Source: three-view drawing plus pictorial views. Frame: mm from the lowest corner of the part. A direction names the side the tool comes from. Give positions to 0.01 mm unless a question says otherwise; leave off trailing zeros. Write each loop counter-clockwise with the first axis right and the second up, starting at its lowest first coordinate (ties: lowest second). Pieces come first, ordered by that corner, then holes.
Q1. Pin query (flat end, axial travel): pin 1 (1.5 mm diameter, centred on x = 1.5, z = 3.5, fed in from -Y); pin 2 (5 mm diameter, centred on x = 2.5, y = 1, fed in from -Z); pin 3 (0.5 mm diameter, centred on y = 4.5, z = 7, fed in from -X). Return the tip coordinate at first contact, or that it passes through.
Q2. Line query: L1, parallel to X at y = 5.5, z = 7.25; L2, parallel to Y at x = 1, z = 1.5; L3, parallel to Y at x = 6, z = 2.5. Output: solid intervals per line, ascending.
Q3. Cut plane D-D on x = 7.5. Return the cut outline in (y, z), plus the area to 3 significant figures.
Q4. Cut plane B-B on y = 5. Return the cut outline in (x, z).
Q5. Cut plane A-A on z = 5. Return the cut outline in (x, y).
Q6. Reachability of the marked faces 1 and 2 from +Z, -Z, +X, -X, +Y, -Y: full face, straight path, thin tool, end or side. Return the list, or none.
Q7. Draft query along Y for the marked faces 3, 4 and 5. Return one class per face: pulls with the +Y half, pulls with the -Y half, needs draft (parallel to the pull), parting line crosses it, or undercut.
Q8. Cut plane C-C on x = 2.75. Return the cut outline in (y, z).
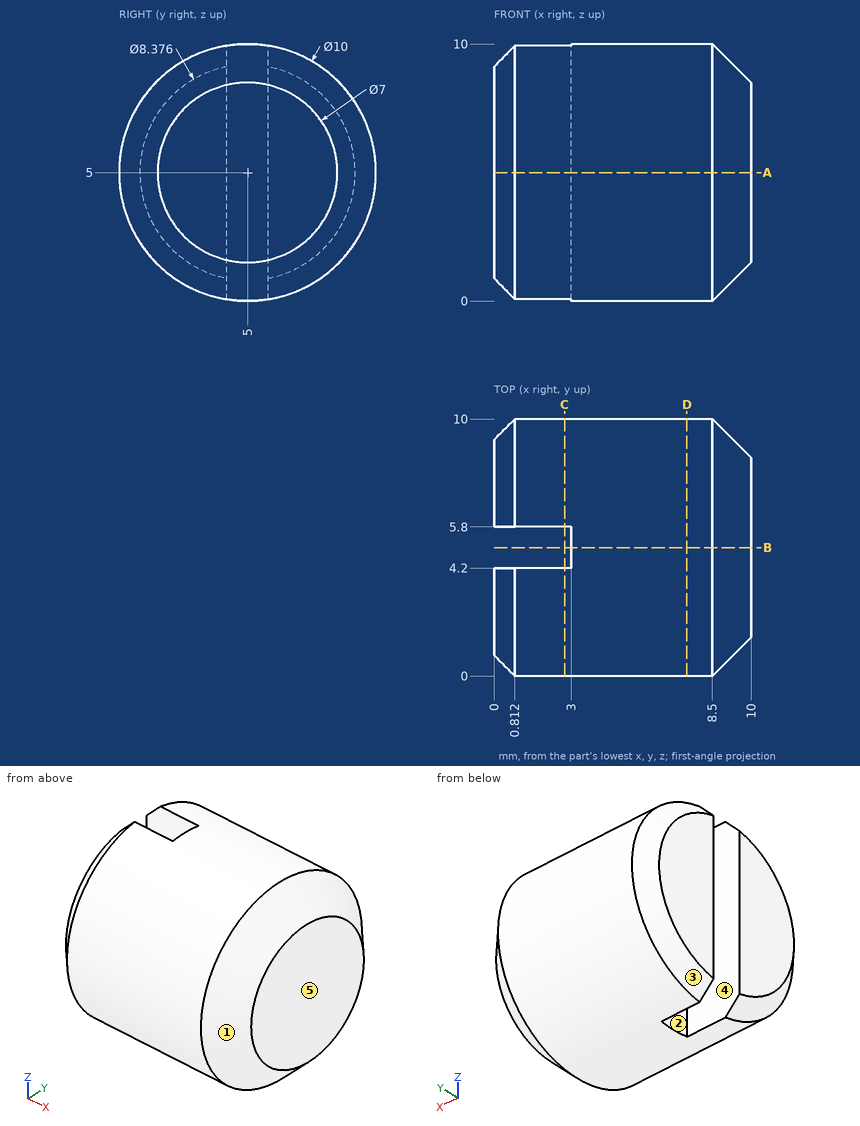
Data:
1. pin 1: stops at y = 0.06
1. pin 2: stops at z = 0.23
1. pin 3: stops at x = 3
2. L1: x = 3 to 10
2. L2: y = 1.43 to 4.2, 5.8 to 8.57
2. L3: y = 0.67 to 9.33
3. outline: circle Ø10 at (5, 5)
3. area: 78.5 mm2
4. outline: (3, 0) - (8.5, 0) - (10, 1.5) - (10, 8.5) - (8.5, 10) - (3, 10) - close
5. outline: (0, 0.81) - (0.81, 0) - (8.5, 0) - (10, 1.5) - (10, 8.5) - (8.5, 10) - (0.81, 10) - (0, 9.19) - (0, 5.8) - (3, 5.8) - (3, 4.2) - (0, 4.2) - close
6. face 1: +X
6. face 2: +Z, -Z, -X
7. face 3: pulls with the +Y half
7. face 4: undercut
7. face 5: needs draft
8. outline: (4.2, 0.06) - (4.2, 9.94) arc R5 ccw to start; (5.8, 0.06) arc R5 ccw to (5.8, 9.94) - close
